Part model, mm, in its own coordinate system. A direction names the side the tool comes from. Coordinates: 2 decimals unless noted, no trailing zeros. Order: outer loops, then holes, each group sorted by start corner. A loop starts at its lowest first (then second) coordinate and runs counter-clockwise, first axis right, second up. Notation, with made-up numbers: (70, 15) - (96, 15) arc R21 ccw to (96, 40) - close; hole circle Ø8 at (-27.75, 49). An arc over 180 degrees is marked (long way). Use a Markdown table: item, result. Add a question column.
1) Wall check: L1, parallel to Z at x = -20, y = 23; L2, parallel to Z at x = -9, y = -27; L3, parallel to X at y = -28, z = 0. Give the ranges that are in metal, low to high. Write a range as [from, to].
2) Saw through at D-D on y = -18.5. List the corners of the cut face in (x, z), then the cut area to 3 significant figures.
3) Saw through at C-C on y = -27. List the corners of the cut face in (x, z), then the cut area to 3 significant figures.
4) Two-plate mould, pull along X, no slides. Class faces 1 (the face through (-8.512, -28.57, 18.196)), 2 (the face through (-19, 5, 0)), 3 (the face through (-24, 3, -7.75)): +X half, -X half, draft (parallel to the pull), parting line (faces both ways), or undercut.
5) Saw through at A-A on y = 23. List the corners of the cut face in (x, z).
6) Tool access for faces 4 (the face through (-30, 0, 15)), 5 (the face through (-13, -28, 0)), 6 (the face through (-24, 4, 7.75)): list every direction of +Z, -Z, +X, -X, +Y, -Y with a clear straight run to the whole face (end or side of a thin tool).
7) Saw through at B-B on z = -10. List the corners of the cut face in (x, y), then the cut area to 3 significant figures.
8) Drop flat-ended pins along their axis: P1, Ø9.5, axis at x = 24, z = 0, coming from the +Y side; P2, Ø2.5, axis at x = 23, z = -16, coming from the +Y side; P3, Ø5, axis at y = 23, z = 6, coming from the +X side; P4, Ø8, axis at x = -9.5, z = -14.5, coming from the -Y side. Give the stop position or say it passes through.
```python
from build123d import *

# Parameters (mm, degrees)
SKETCH1_W                  = 62
SKETCH1_H                  = 67
BOSS_EXTRUDE1_DEPTH        = 20
SKETCH2_W                  = 50
SKETCH2_H                  = 57
CUT_EXTRUDE1_DEPTH         = 61.689784972
SKETCH3_W                  = 2
SKETCH3_H                  = 30
CUT_EXTRUDE2_DEPTH         = 77.485292704
CUT_EXTRUDE3_DEPTH         = 64.421210963
F_4_5_4_5_DIAMETER_HOLE1_D = 4.5
SKETCH7_R                  = 3
CUT_EXTRUDE4_DEPTH         = 68.896980787
CHAMFER1_SIZE              = 3
CUT_EXTRUDE5_DEPTH         = 68.896980787


with BuildPart() as part:
    # Sketch1 → Boss-Extrude1 (new, symmetric)
    with BuildSketch(Plane.XY):
        Rectangle(SKETCH1_W, SKETCH1_H)
    extrude(amount=BOSS_EXTRUDE1_DEPTH, both=True)

    # Sketch2 → Cut-Extrude1 (cut, through all)
    with BuildSketch(Plane.XY.offset(20)):
        with Locations((6, 5)):
            Rectangle(SKETCH2_W, SKETCH2_H)
    extrude(amount=-CUT_EXTRUDE1_DEPTH, mode=Mode.SUBTRACT)

    # Sketch3 → Cut-Extrude2 (cut, through all)
    with BuildSketch(Plane(origin=(0, 33.5, 0), x_dir=(1, 0, 0), z_dir=(0, 1, 0))):
        with Locations((-30, 0)):
            Rectangle(SKETCH3_W, SKETCH3_H)
    extrude(amount=-CUT_EXTRUDE2_DEPTH, mode=Mode.SUBTRACT)

    # Sketch4 → Cut-Extrude3 (cut, through all)
    with BuildSketch(Plane(origin=(-19, 0, 0), x_dir=(0, 0, -1), z_dir=(1, 0, 0))):
        with BuildLine():
            Line((-7.75, 26.5), (-7.75, 20.5))
            ThreePointArc((-7.75, 20.5), (-10, 18.25), (-12.25, 20.5))
            Line((-12.25, 20.5), (-12.25, 26.5))
            ThreePointArc((-12.25, 26.5), (-10, 28.75), (-7.75, 26.5))
        make_face()
        with BuildLine():
            Line((-7.75, 6.5), (-7.75, 0.5))
            ThreePointArc((-7.75, 0.5), (-10, -1.75), (-12.25, 0.5))
            Line((-12.25, 0.5), (-12.25, 6.5))
            ThreePointArc((-12.25, 6.5), (-10, 8.75), (-7.75, 6.5))
        make_face()
        with BuildLine():
            Line((12.25, 26.5), (12.25, 20.5))
            ThreePointArc((12.25, 20.5), (10, 18.25), (7.75, 20.5))
            Line((7.75, 20.5), (7.75, 26.5))
            ThreePointArc((7.75, 26.5), (10, 28.75), (12.25, 26.5))
        make_face()
        with BuildLine():
            Line((12.25, 6.5), (12.25, 0.5))
            ThreePointArc((12.25, 0.5), (10, -1.75), (7.75, 0.5))
            Line((7.75, 0.5), (7.75, 6.5))
            ThreePointArc((7.75, 6.5), (10, 8.75), (12.25, 6.5))
        make_face()
    extrude(amount=-CUT_EXTRUDE3_DEPTH, mode=Mode.SUBTRACT)

    # Ø4.5 (4.5) Diameter Hole1 (through all)
    with Locations(Plane(origin=(0, -23.5, 0), x_dir=(1, 0, 0), z_dir=(0, 1, 0))):
        with Locations((-9, 16), (-9, -16), (23, -16), (23, 16)):
            Hole(F_4_5_4_5_DIAMETER_HOLE1_D / 2)

    # Sketch7 → Cut-Extrude4 (cut, through all)
    with BuildSketch(Plane(origin=(0, -23.5, 0), x_dir=(1, 0, 0), z_dir=(0, 1, 0))):
        with Locations(Location((24, 0, 0), (0, 0, 270))):
            Circle(SKETCH7_R)
        with BuildLine():
            Line((-10, 3), (-8, 3))
            ThreePointArc((-8, 3), (-5, 0), (-8, -3))
            Line((-8, -3), (-10, -3))
            ThreePointArc((-10, -3), (-13, 0), (-10, 3))
        make_face()
    extrude(amount=-CUT_EXTRUDE4_DEPTH, mode=Mode.SUBTRACT)

    # Chamfer1
    chamfer1_edges = [part.edges().sort_by_distance(p)[0] for p in [
        (-25, 33.5, -20),
        (-25, 33.5, 20),
        (31, -28.5, 20),
        (31, -28.5, -20),
    ]]
    chamfer(chamfer1_edges, length=CHAMFER1_SIZE)

    # Sketch8 → Cut-Extrude5 (cut, through all)
    with BuildSketch(Plane(origin=(0, -23.5, 0), x_dir=(1, 0, 0), z_dir=(0, 1, 0))):
        with BuildLine():
            Line((6.25, -19.5), (6.25, -27.0274699))
            ThreePointArc((6.25, -27.0274699), (2, -31.2774699), (-2.25, -27.0274699))
            Line((-2.25, -27.0274699), (-2.25, -19.5))
            ThreePointArc((-2.25, -19.5), (2, -15.25), (6.25, -19.5))
        make_face()
        with BuildLine():
            Line((-2.25, 19.5), (-2.25, 27.0274699))
            ThreePointArc((-2.25, 27.0274699), (2, 31.2774699), (6.25, 27.0274699))
            Line((6.25, 27.0274699), (6.25, 19.5))
            ThreePointArc((6.25, 19.5), (2, 15.25), (-2.25, 19.5))
        make_face()
    extrude(amount=-CUT_EXTRUDE5_DEPTH, mode=Mode.SUBTRACT)


solid = part.part
```
Results are:
| question | item | result |
|---|---|---|
| 1 | L1 | [-20, -12.25], [-7.75, 7.75], [12.25, 20] |
| 1 | L2 | [-20, -18.25], [-13.75, -3], [3, 13.75], [18.25, 20] |
| 1 | L3 | [-29, -13], [-5, 21], [27, 31] |
| 2 | outline | (-31, -20) - (-19, -20) - (-19, 20) - (-31, 20) - (-31, 15) - (-29, 15) - (-29, -15) - (-31, -15) - close |
| 2 | area | 420 mm2 |
| 3 | outline | (-31, -20) - (-2.25, -20) - (-2.25, -19.5) arc R4.25 cw to (6.25, -19.5) - (6.25, -20) - (28, -20) - (31, -17) - (31, 17) - (28, 20) - (6.25, 20) - (6.25, 19.5) arc R4.25 cw to (-2.25, 19.5) - (-2.25, 20) - (-31, 20) - (-31, 15) - (-29, 15) - (-29, -15) - (-31, -15) - close; hole circle Ø4.5 at (-9, -16); hole circle Ø4.5 at (-9, 16); hole (-10, -3) - (-8, -3) arc R3 ccw to (-8, 3) - (-10, 3) arc R3 ccw to start; hole circle Ø4.5 at (23, -16); hole circle Ø4.5 at (23, 16); hole circle Ø6 at (24, 0) |
| 3 | area | 2,210 mm2 |
| 4 | face 1 | undercut |
| 4 | face 2 | +X half |
| 4 | face 3 | draft |
| 5 | outline | (-31, -20) - (-19, -20) - (-19, -12.25) - (-29, -12.25) - (-29, -15) - (-31, -15) - close; (-31, 15) - (-29, 15) - (-29, 12.25) - (-19, 12.25) - (-19, 20) - (-31, 20) - close; (-29, -7.75) - (-19, -7.75) - (-19, 7.75) - (-29, 7.75) - close |
| 6 | face 4 | -X, +Y, -Y |
| 6 | face 5 | +Y, -Y |
| 6 | face 6 | +X, -X |
| 7 | outline | (-29, -33.5) - (31, -33.5) - (31, -23.5) - (-19, -23.5) - (-19, -1.75) - (-29, -1.75) - close; (-29, 8.75) - (-19, 8.75) - (-19, 18.25) - (-29, 18.25) - close; (-29, 28.75) - (-19, 28.75) - (-19, 33.5) - (-29, 33.5) - close |
| 7 | area | 960 mm2 |
| 8 | P1 | y = -23.5 |
| 8 | P2 | through |
| 8 | P3 | x = -19 |
| 8 | P4 | y = -33.5 |
